Verification items for the finished model (mm, model axes). A direction names the side the tool comes from. Coordinates: 2 decimals unless noted, no trailing zeros. Write each loop counter-clockwise with the first axis right and the second up, starting at its lowest first coordinate (ties: lowest second). Pieces come first, ordered by that corner, then holes. Notation, with made-up numbers: M -10.5,48.25 L 23.5,48.25 A27 ccw 23.5,81.25 Z; hole C 51.5,-5 d5. An arc over 180 degrees is marked long. One line per item, written item: value.
```python
from build123d import *

# Parameters (mm, degrees)
H_BODY_EXTRUDE_60_DEPTH   = 60
RELIEF_CUT_10_DEPTH       = 10
CONNECTOR_ARM_SKETCH_R    = 7.5
CONNECTOR_ARM_BOSS_DEPTH  = 10
NOTCH_CUT_A_SKETCH_W      = 60
NOTCH_CUT_A_SKETCH_H      = 40
NOTCH_CUT_A_DEPTH         = 10
NOTCH_CUT_B_SKETCH_W      = 60
NOTCH_CUT_B_SKETCH_H      = 40
NOTCH_CUT_B_DEPTH         = 10
LINK_PLATE_SKETCH_R       = 7.5
LINK_PLATE_BOSS_DEPTH     = 10
LINK_PLATE_HOLES_SKETCH_W = 50
LINK_PLATE_HOLES_SKETCH_H = 15
LINK_PLATE_HOLES_DEPTH    = 105.880884817
EDGE_FILLETS_R5_R         = 5


with BuildPart() as part:
    # H Profile Sketch → H Body Extrude 60 (new body)
    with BuildSketch(Plane.XY):
        Polygon((0, 0), (0, 45), (10, 45), (10, 5), (50, 5), (50, 45), (60, 45), (60, -45), (50, -45), (50, -5), (10, -5), (10, -45), (0, -45), align=None)
    extrude(amount=H_BODY_EXTRUDE_60_DEPTH)

    # Relief Cut Sketch → Relief Cut 10 (cut)
    with BuildSketch(Plane.ZY):
        with BuildLine():
            Line((10, 35), (0, 35))
            Line((0, 35), (0, 15))
            Line((0, 15), (10, 15))
            ThreePointArc((10, 15), (20, 25), (10, 35))
        make_face()
        with BuildLine():
            Line((60, 15), (60, 35))
            Line((60, 35), (50, 35))
            ThreePointArc((50, 35), (40, 25), (50, 15))
            Line((50, 15), (60, 15))
        make_face()
        with BuildLine():
            Line((10, -15), (0, -15))
            Line((0, -15), (0, -35))
            Line((0, -35), (10, -35))
            ThreePointArc((10, -35), (20, -25), (10, -15))
        make_face()
        with BuildLine():
            Line((60, -35), (60, -15))
            Line((60, -15), (50, -15))
            ThreePointArc((50, -15), (40, -25), (50, -35))
            Line((50, -35), (60, -35))
        make_face()
    extrude(amount=-RELIEF_CUT_10_DEPTH, mode=Mode.SUBTRACT)

    # Connector Arm Sketch → Connector Arm Boss (add)
    with BuildSketch(Plane(origin=(60, 0, 0), x_dir=(0, 0, -1), z_dir=(1, 0, 0))):
        with BuildLine():
            Line((-15, 30), (-15, -30))
            ThreePointArc((-15, -30), (-30, -45), (-45, -30))
            Line((-45, -30), (-45, 30))
            ThreePointArc((-45, 30), (-30, 45), (-15, 30))
        make_face()
        with Locations((-30, 30)):
            Circle(CONNECTOR_ARM_SKETCH_R, mode=Mode.SUBTRACT)
        with Locations((-30, -30)):
            Circle(CONNECTOR_ARM_SKETCH_R, mode=Mode.SUBTRACT)
    extrude(amount=-CONNECTOR_ARM_BOSS_DEPTH)

    # Notch Cut A Sketch → Notch Cut A (cut)
    with BuildSketch(Plane.ZY.offset(-50)):
        with Locations((30, 25)):
            Rectangle(NOTCH_CUT_A_SKETCH_W, NOTCH_CUT_A_SKETCH_H)
    extrude(amount=-NOTCH_CUT_A_DEPTH, mode=Mode.SUBTRACT)

    # Notch Cut B Sketch → Notch Cut B (cut)
    with BuildSketch(Plane.ZY.offset(-50)):
        with Locations((30, -25)):
            Rectangle(NOTCH_CUT_B_SKETCH_W, NOTCH_CUT_B_SKETCH_H)
    extrude(amount=-NOTCH_CUT_B_DEPTH, mode=Mode.SUBTRACT)

    # Link Plate Sketch → Link Plate Boss (add)
    with BuildSketch(Plane(origin=(60, 0, 0), x_dir=(0, 0, -1), z_dir=(1, 0, 0))):
        with BuildLine():
            Line((-15, 30), (-15, -30))
            ThreePointArc((-15, -30), (-30, -45), (-45, -30))
            Line((-45, -30), (-45, 30))
            ThreePointArc((-45, 30), (-30, 45), (-15, 30))
        make_face()
        with Locations((-30, 30)):
            Circle(LINK_PLATE_SKETCH_R, mode=Mode.SUBTRACT)
        with Locations((-30, -30)):
            Circle(LINK_PLATE_SKETCH_R, mode=Mode.SUBTRACT)
    extrude(amount=LINK_PLATE_BOSS_DEPTH)

    # Link Plate Holes Sketch → Link Plate Holes (cut, through all)
    with BuildSketch(Plane(origin=(0, 5, 0), x_dir=(1, 0, 0), z_dir=(0, 1, 0))):
        with Locations((35, -7.5)):
            Rectangle(LINK_PLATE_HOLES_SKETCH_W, LINK_PLATE_HOLES_SKETCH_H)
        with Locations((35, -52.5)):
            Rectangle(LINK_PLATE_HOLES_SKETCH_W, LINK_PLATE_HOLES_SKETCH_H)
    extrude(amount=-LINK_PLATE_HOLES_DEPTH, mode=Mode.SUBTRACT)

    # Edge Fillets R5
    edge_fillets_r5_edges = [part.edges().sort_by_distance(p)[0] for p in [
        (10, 0, 15),
        (10, 0, 45),
    ]]
    fillet(edge_fillets_r5_edges, radius=EDGE_FILLETS_R5_R)


solid = part.part
```
Item 1: Draft check along X on faces 1 (the face through (70, 1, 30)), 2 (the face through (5, 15, 55)), 3 (the face through (10, 11, 30)). Enter one of: released by +X, released by -X, zero draft, split by the parting line, or undercut.
The answers:
face 1: released by +X
face 2: zero draft
face 3: undercut
Item 2: Access from +Z, -Z, +X, -X, +Y, -Y to the whole of each face (thin tool, end or side, straight path). Record for faces 4 (the face through (5, -25, 20)), 5 (the face through (64.93, 22.68, 31.63)), 6 (the face through (5, 35, 5)), 7 (the face through (5, -25, 40)), 8 (the face through (5, 35, 55)).
The answers:
face 4: -Z, -X
face 5: +X
face 6: -Z, +X, -X
face 7: +Z, -X
face 8: +Z, +X, -X
Item 3: Cross-section at C-C, the plane y = -33. Enter the section's corners in (x, z).
The answers:
outline: M 0,16 L 10,16 L 10,44 L 0,44 Z; M 60,15.3 L 70,15.3 L 70,23.13 L 60,23.13 Z; M 60,36.87 L 70,36.87 L 70,44.7 L 60,44.7 Z
Item 4: Scan lines: line 1 (Y direction, x = 64, z = 30); line 2 (X direction, y = 9, z = 37); line 3 (Y direction, x = 6.5, z = 58). Record each from-to range of solid material in increasing order.
The answers:
line 1: y = -45 to -37.5, -22.5 to 22.5, 37.5 to 45
line 2: x = 0 to 10, 60 to 70
line 3: y = -45 to -35, -15 to 15, 35 to 45
Item 5: Cross-section at B-B, the plane x = 5.5. Enter the section's corners in (y, z).
The answers:
outline: M -45,0 L -35,0 L -35,10 A10 cw -15,10 L -15,0 L 15,0 L 15,10 A10 cw 35,10 L 35,0 L 45,0 L 45,60 L 35,60 L 35,50 A10 cw 15,50 L 15,60 L -15,60 L -15,50 A10 cw -35,50 L -35,60 L -45,60 Z
Item 6: Cross-section at A-A, the plane z = 18. Enter the section's corners in (x, y).
The answers:
outline: M 0,-45 L 10,-45 L 10,-31 L 0,-31 Z; M 0,-19 L 10,-19 L 10,-5 L 60,-5 L 60,-39 L 70,-39 L 70,39 L 60,39 L 60,5 L 10,5 L 10,19 L 0,19 Z; M 0,31 L 10,31 L 10,45 L 0,45 Z
Item 7: Cross-section at D-D, the plane z = 30. Enter the section's corners in (x, y), and give its area (3 significant figures).
The answers:
outline: M 0,-45 L 10,-45 L 10,-5 L 60,-5 L 60,-22.5 L 70,-22.5 L 70,22.5 L 60,22.5 L 60,5 L 10,5 L 10,45 L 0,45 Z; M 60,-45 L 70,-45 L 70,-37.5 L 60,-37.5 Z; M 60,37.5 L 70,37.5 L 70,45 L 60,45 Z
area: 2,000 mm²
Item 8: Go/stop test with flat-tipped pins: P1, Ø12, axis at x = 39.5, z = 32.5, coming from the +Y side; P2, Ø1.5, axis at x = 55, z = 38, coming from the -Y side; P3, Ø2, axis at x = 63, y = 23.5, coming from the +Z side. Record where each tip stops, or that it passes through.
The answers:
P1: stops at y = 5
P2: stops at y = -5
P3: stops at z = 45
